Read the model definition and answer for the solid it produces. Units are mm, in the model's axes. Round coordinates to 2 decimals unless told otherwise and drop trailing zeros. Loops run counter-clockwise (first coordinate to the right, second up) from the corner with the lowest first, then second, coordinate; pieces in that order, holes last. Notation, with made-up numbers: (84.25, 78) - (104.25, 78) arc R4 ccw to (104.25, 83) - close; hole circle Ø2 at (15, -17). An arc over 180 degrees is marked (long way). Use one line per item in the form item = value. Start each with the question number.
```python
from build123d import *

# Parameters (mm, degrees)
SKETCH1_R                  = 450
SKETCH1_R_2                = 340
BOSS_EXTRUDE1_DEPTH        = 4
F_15_0_15_DIAMETER_HOLE1_D = 15


with BuildPart() as part:
    # Sketch1 → Boss-Extrude1 (new, symmetric)
    with BuildSketch(Plane(origin=(0, 0, 0), x_dir=(1, 0, 0), z_dir=(0, 1, 0))):
        with Locations(Location((0, 0, 0), (0, 0, 270))):
            Circle(SKETCH1_R)
        with Locations(Location((0, 0, 0), (0, 0, 270))):
            Circle(SKETCH1_R_2, mode=Mode.SUBTRACT)
    extrude(amount=BOSS_EXTRUDE1_DEPTH, both=True)

    # Ø15.0 (15) Diameter Hole1 (through all)
    with Locations(Plane(origin=(0, 4, 0), x_dir=(1, 0, 0), z_dir=(0, 1, 0))):
        with Locations((153.073372946, 369.551813005), (369.551813005, 153.073372946), (369.551813005, -153.073372946), (153.073372946, -369.551813005), (-153.073372946, -369.551813005), (-369.551813005, -153.073372946), (-369.551813005, 153.073372946), (-153.073372946, 369.551813005)):
            Hole(F_15_0_15_DIAMETER_HOLE1_D / 2)


solid = part.part
```
1) Straight lines are drawn through the part: line 1 (X direction, y = -0.75, z = 0); line 2 (Z direction, x = -367.5, y = -0.5); line 3 (Z direction, x = 175, y = 3.5). For each, find the intervals that lie inside material, in ascending order. Write a range as from..to.
2) A cutting plane is placed at A-A on x = 0. Write down the section's boundary in (y, z).
3) Determine the mould class of faces 1 (the cylindrical face through (-206.9, -0.1, -269.8)), 2 (the cylindrical face through (19.786, 0.056, -449.565)), 3 (the flat face through (335, 4, 65)) for opening direction X: +X half, -X half, draft (parallel to the pull), parting line (faces both ways), or undercut.
4) Flat-ended cylindrical pins translate along their axes: pin 1 (12 mm diameter, centred on x = -369.55, z = -153.07, fed in from +Y); pin 2 (17 mm diameter, centred on x = -153.07, z = 369.55, fed in from +Y); pin 3 (3 mm diameter, centred on y = 1, z = -132.5, fed in from +X); pin 4 (4 mm diameter, centred on y = 0, z = 196, fed in from -X). Find the tip coordinate at first contact, or state that the pin passes through.
5) A cutting plane is placed at B-B on z = -86. Write down the section's boundary in (x, y), plus the area to 3 significant figures.
6) A cutting plane is placed at C-C on y = 2.75. Count the separate pieces of the cut face and the enclosed holes in it, plus the area to 3 significant figures.
Checks:
q1.line_1 = -450..-340, 340..450
q1.line_2 = -259.7..-160.29, -145.86..145.86, 160.29..259.7
q1.line_3 = -414.58..-291.5, 291.5..414.58
q2.outline = (-4, -450) - (4, -450) - (4, -340) - (-4, -340) - close; (-4, 340) - (4, 340) - (4, 450) - (-4, 450) - close
q3.face_1 = undercut
q3.face_2 = parting line
q3.face_3 = draft
q4.pin_1 = through
q4.pin_2 = 4
q4.pin_3 = 430.51
q4.pin_4 = -406.03
q5.outline = (-441.71, -4) - (-328.94, -4) - (-328.94, 4) - (-441.71, 4) - close; (328.94, -4) - (441.71, -4) - (441.71, 4) - (328.94, 4) - close
q5.area = 1,800 mm²
q6.separate_pieces = 1
q6.enclosed_holes = 9
q6.area = 272,000 mm²
